```python
from build123d import *

# Parameters (mm, degrees)
EXTRUDE_1_DEPTH             = 12
HOLE_WIZARD_8_5_8_5_1_D     = 8.5
HOLE_WIZARD_8_5_8_5_1_DEPTH = 15.61
HOLE_WIZARD_8_5_8_5_1_TIP   = 2.453738644
SKETCH_5_R                  = 4
CUT_EXTRUDE_1_DEPTH         = 12
HOLE_WIZARD_M6_1_D          = 5
HOLE_WIZARD_M6_1_DEPTH      = 25
CHAMFER_1_SIZE              = 1
CHAMFER_2_SIZE              = 1


with BuildPart() as part:
    # 草图1 → 凸台-拉伸1 (new body)
    with BuildSketch(Plane.XY):
        Polygon((74.869050236, -20), (4.869050236, -20), (4.869050236, 0), (49.869050236, 67.029820029), (49.869050236, 171), (0.869050236, 171), (0.869050236, 196), (74.869050236, 196), align=None)
    extrude(amount=-EXTRUDE_1_DEPTH)

    # Ø8.5 (8.5) 直径孔1
    with Locations(Plane.XY):
        with Locations((64.869050236, -10), (14.869050236, -10)):
            Hole(HOLE_WIZARD_8_5_8_5_1_D / 2, depth=HOLE_WIZARD_8_5_8_5_1_DEPTH)
            with Locations((0, 0, -(HOLE_WIZARD_8_5_8_5_1_DEPTH + HOLE_WIZARD_8_5_8_5_1_TIP / 2))):  # 120° drill point
                Cone(0, HOLE_WIZARD_8_5_8_5_1_D / 2, HOLE_WIZARD_8_5_8_5_1_TIP, mode=Mode.SUBTRACT)

    # 草图5 → 切除-拉伸1 (cut)
    with BuildSketch(Plane.XY):
        with Locations((29.869050236, -10)):
            Circle(SKETCH_5_R)
        with Locations((49.869050236, -10)):
            Circle(SKETCH_5_R)
    extrude(amount=-CUT_EXTRUDE_1_DEPTH, mode=Mode.SUBTRACT)

    # M6 螺纹孔1
    with Locations(Plane(origin=(0, 196, 0), x_dir=(1, 0, 0), z_dir=(0, 1, 0))):
        with Locations((10.869050236, 6), (30.869050236, 6)):
            Hole(HOLE_WIZARD_M6_1_D / 2, depth=HOLE_WIZARD_M6_1_DEPTH)

    # 倒角1
    chamfer_1_edges = [part.edges().sort_by_distance(p)[0] for p in [
        (74.869050236, -20, -6),
        (74.869050236, 196, -6),
    ]]
    chamfer(chamfer_1_edges, length=CHAMFER_1_SIZE)

    # 倒角2
    chamfer_2_edges = [part.edges().sort_by_distance(p)[0] for p in [
        (4.869050236, -20, -6),
    ]]
    chamfer(chamfer_2_edges, length=CHAMFER_2_SIZE)


solid = part.part
```
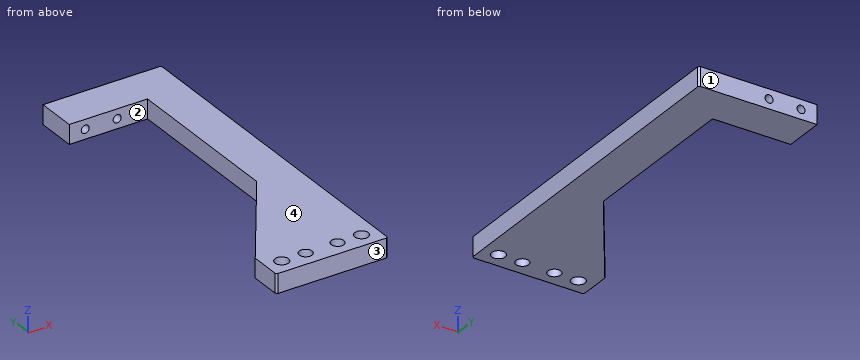
Geometry: final body of the model. Coordinates: model frame, mm. Face numbers are marked on the shaded views. Give positions to 0.01 mm unless a question says otherwise; leave off trailing zeros. Order: outer loops, then holes, each group sorted by start corner. A loop starts at its lowest first (then second) coordinate and runs counter-clockwise, first axis right, second up. Notation, with made-up numbers: (70, 76) -> (122, 76) arc R6 ccw to (122, 85) -> close; hole circle Ø1 at (9, 56.25). An arc over 180 degrees is marked (long way). Write each question's results on one line, items separated by ' | '. Start each with the question number.
1) Section D-D (y = 181). Return loops of the section in (x, z), then the cut area to 3 significant figures.
2) First-contact query: pin 1 (3.5 mm diameter, centred on y = -9.5, z = -7, fed in from -X); pin 2 (3.5 mm diameter, centred on y = 115, z = -7.5, fed in from -X); pin 3 (5 mm diameter, centred on x = 29.87, y = -10, fed in from +Z). Flat tips, straight axial feed; report the tip coordinate or a pass-through.
3) Line query: line 1 (Y direction, x = 47, z = -1.5); line 2 (Y direction, x = 49, z = -7.5); line 3 (Y direction, x = 34.5, z = -5.75). Output: solid intervals per line, ascending. Write a range as from..to.
4) Section B-B (z = -6). Return loops of the section in (x, y).
5) Section C-C (x = 40.5). Return loops of the section in (y, z).
6) Draft query along Y for the marked faces 1, 2, 3 and 4. Return one class per face: pulls with the +Y half, pulls with the -Y half, needs draft (parallel to the pull), parting line crosses it, or undercut.
7) Section A-A (y = -10). Return loops of the section in (x, z).
Calculated:
1) outline: (0.87, -12) -> (74.87, -12) -> (74.87, 0) -> (0.87, 0) -> close; hole circle Ø5 at (10.87, -6); hole circle Ø5 at (30.87, -6) | area: 849 mm2
2) pin 1: x = 4.87 | pin 2: x = 49.87 | pin 3: through
3) line 1: -20..-12.79, -7.21..62.76, 171..196 | line 2: -20..-13.9, -6.1..65.74, 171..196 | line 3: -20..44.14, 171..196
4) outline: (0.87, 171) -> (8.37, 171) -> (8.37, 196) -> (0.87, 196) -> close; (4.87, -19) -> (5.87, -20) -> (73.87, -20) -> (74.87, -19) -> (74.87, 195) -> (73.87, 196) -> (33.37, 196) -> (33.37, 171) -> (49.87, 171) -> (49.87, 67.03) -> (4.87, 0) -> close; (13.37, 171) -> (28.37, 171) -> (28.37, 196) -> (13.37, 196) -> close; hole circle Ø8.5 at (14.87, -10); hole circle Ø8 at (29.87, -10); hole circle Ø8 at (49.87, -10); hole circle Ø8.5 at (64.87, -10)
5) outline: (-20, -12) -> (53.07, -12) -> (53.07, 0) -> (-20, 0) -> close; (171, -12) -> (196, -12) -> (196, 0) -> (171, 0) -> close
6) face 1: pulls with the +Y half | face 2: undercut | face 3: pulls with the -Y half | face 4: needs draft
7) outline: (4.87, -12) -> (10.62, -12) -> (10.62, 0) -> (4.87, 0) -> close; (19.12, -12) -> (25.87, -12) -> (25.87, 0) -> (19.12, 0) -> close; (33.87, -12) -> (45.87, -12) -> (45.87, 0) -> (33.87, 0) -> close; (53.87, -12) -> (60.62, -12) -> (60.62, 0) -> (53.87, 0) -> close; (69.12, -12) -> (74.87, -12) -> (74.87, 0) -> (69.12, 0) -> close
